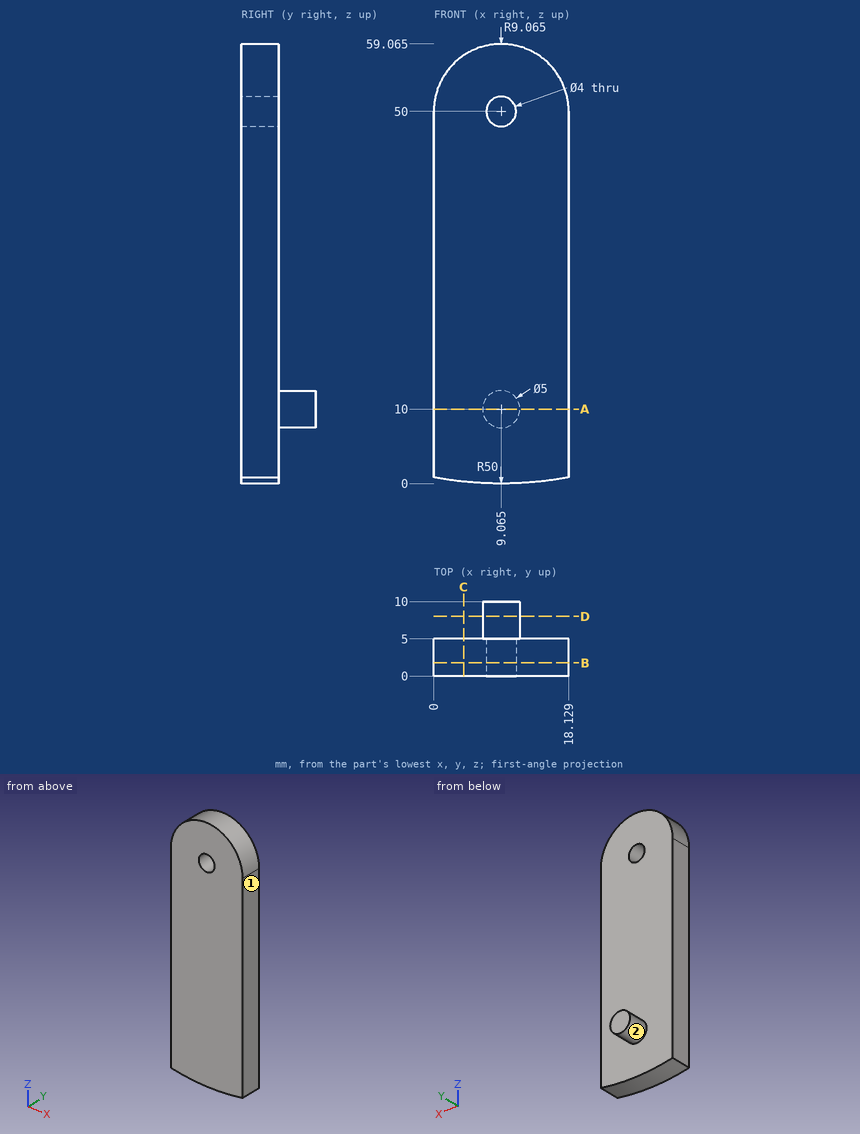
Here's the drawing with two shaded views (mm, measured from the low corner). I have some questions. A direction names the side the tool comes from. Round coordinates to 2 decimals unless told otherwise and drop trailing zeros. Loops run counter-clockwise (first coordinate to the right, second up) from the corner with the lowest first, then second, coordinate; pieces in that order, holes last. Notation, with made-up numbers: M -33.5,-35.5 L -26.5,-35.5 A25 ccw -26.5,-2.5 Z; hole C 15.25,77.5 d5. An arc over 180 degrees is marked long. Answer as a JSON object with one key per item and string values. Group by question number.
Q1. Imagine slicing it at B-B, the plane y = 1.75. Please give me the cut outline in (x, z) (1 decimal).
Q2. Imagine slicing it at C-C, the plane x = 4. Please give me the cut outline in (y, z), then the cut area to 3 significant figures.
Q3. Please list where these lines run through material, in increasing order: L1, parallel to X at y = 2.45, z = 50 (1 decimal); L2, parallel to Y at x = 16.25, z = 52.5; L3, parallel to Z at x = 9.25, y = 2.5.
Q4. Will these pins go through, and if not, where does the flat tip stop? pin 1 (10 mm diameter, centred on x = 4.5, z = 23, fed in from +Y); pin 2 (5 mm diameter, centred on x = 15, y = 6, fed in from +Z); pin 3 (6 mm diameter, centred on x = 13.5, y = 8.5, fed in from -Z).
Q5. Imagine slicing it at D-D, the plane y = 8. Please give me the cut outline in (x, z) (1 decimal).
Q6. Imagine slicing it at A-A, the plane z = 10. Please give me the cut outline in (x, y) (1 decimal), then the cut area to 3 significant figures.
Q7. On a 3-axis mill with a long thin cutter (end or side, diameter ignored), from which of +Z, -Z, +X, -X, +Y, -Y can I reach the whole of each face in a straight line? I mean the marked faces 1 and 2. Say none if no direction works.
Findings:
{
 "1": {"outline": "M 0,0.8 A50 ccw 18.1,0.8 L 18.1,50 A9.1 ccw 0,50 Z; hole C 9.1,50 d4"},
 "2": {"outline": "M 0,0.26 L 5,0.26 L 5,57.52 L 0,57.52 Z", "area": "286 mm2"},
 "3": {"L1": "x = 0 to 7.1, 11.1 to 18.1", "L2": "y = 0 to 5", "L3": "z = 0 to 48.01, 51.99 to 59.06"},
 "4": {"pin 1": "stops at y = 5", "pin 2": "stops at z = 58.3", "pin 3": "stops at z = 7.95"},
 "5": {"outline": "C 9.1,10 d5"},
 "6": {"outline": "M 0,0 L 18.1,0 L 18.1,5 L 11.6,5 L 11.6,10 L 6.6,10 L 6.6,5 L 0,5 Z", "area": "116 mm2"},
 "7": {"face 1": "+Z, -Z, +X, +Y, -Y", "face 2": "+Y"}
}
